Part print with two shaded views. Sizes in mm from the minimum x, y, z corner. Round coordinates to 2 decimals unless told otherwise and drop trailing zeros.
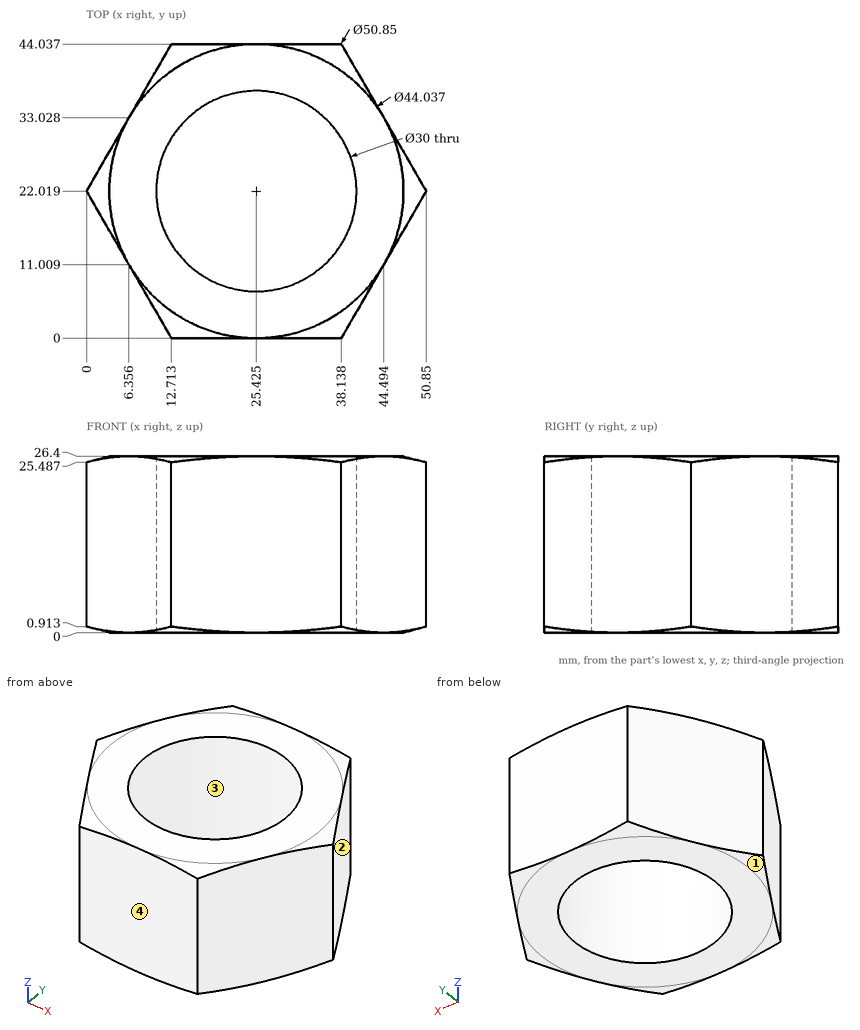
Q1. Drop flat-ended pins along their axis: pin 1 (4 mm diameter, centred on y = 30, z = 6, fed in from +X); pin 2 (8 mm diameter, centred on y = 38.5, z = 20, fed in from -X) (1 decimal); pin 3 (3 mm diameter, centred on y = 10.5, z = 13, fed in from +X) (1 decimal). Give the stop position or say it passes through.
Values follow:
pin 1: stops at x = 47.4
pin 2: stops at x = 7.2
pin 3: stops at x = 45.1
Q2. Mould opens along Y. For the marked faces 1, 2, 3 and 4 say: +Y half, -Y half, draft (parallel to the pull), parting line (faces both ways), or undercut.
Values follow:
face 1: parting line
face 2: +Y half
face 3: undercut
face 4: -Y half
Q3. Wall check: L1, parallel to X at y = 30, z = 12.25 (1 decimal); L2, parallel to X at y = 9, z = 2.25 (1 decimal); L3, parallel to Y at x = 12.5, z = 1.5 (1 decimal). Give the ranges that are in metal, low to high.
Values follow:
L1: x = 4.6 to 12.7, 38.1 to 46.2
L2: x = 7.5 to 18, 32.9 to 43.3
L3: y = 0.4 to 14.4, 29.6 to 43.7
